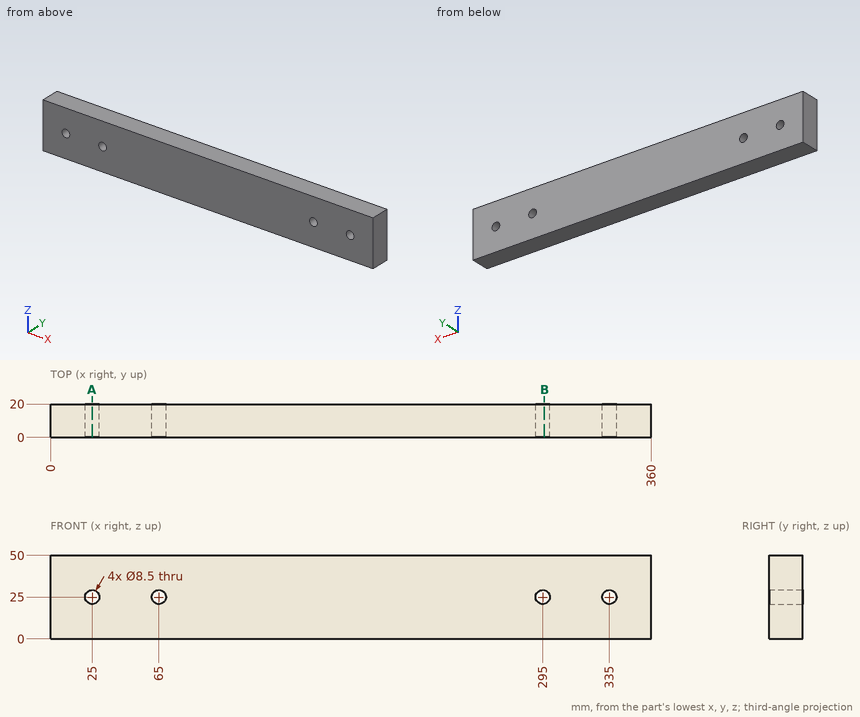
Input: dimensioned drawing with shaded views. Units: mm. Origin: part minimum x, y, z. Coordinates: 2 decimals unless noted, no trailing zeros. Loops run counter-clockwise (first coordinate to the right, second up) from the corner with the lowest first, then second, coordinate; pieces in that order, holes last. Notation, with made-up numbers: (-6, 36.5) -> (40, 36.5) arc R24 ccw to (40, 72.5) -> close; hole circle Ø4 at (15.25, 9.25). An arc over 180 degrees is marked (long way). One line per item, written item: value. Start each with the question number.
Q1. Contact query for a flat-ended pin moving along its axis: P1, Ø5, axis at x = 335, z = 25, coming from the +Y side. Output: stop coordinate, or through.
Q2. Section query A-A, the plane x = 25. Return the cut outline in (y, z), and give its area (3 significant figures).
Q3. Section query B-B, the plane x = 296. Return the cut outline in (y, z), and give its area (3 significant figures).
Q4. Line query: line 1 along X through (y, z) = (12.5, 25); line 2 along Z through (x, y) = (295, 6.75). Output: solid intervals per line, ascending.
Results:
1. P1: through
2. outline: (0, 0) -> (20, 0) -> (20, 20.75) -> (0, 20.75) -> close; (0, 29.25) -> (20, 29.25) -> (20, 50) -> (0, 50) -> close
2. area: 830 mm^2
3. outline: (0, 0) -> (20, 0) -> (20, 20.87) -> (0, 20.87) -> close; (0, 29.13) -> (20, 29.13) -> (20, 50) -> (0, 50) -> close
3. area: 835 mm^2
4. line 1: 0 to 20.75, 29.25 to 60.75, 69.25 to 290.75, 299.25 to 330.75, 339.25 to 360
4. line 2: 0 to 20.75, 29.25 to 50
